Build history of the part. All positions in model axes, mm. A direction names the side the tool comes from. Round coordinates to 2 decimals unless told otherwise and drop trailing zeros. Write each loop counter-clockwise with the first axis right and the second up, starting at its lowest first coordinate (ties: lowest second). Pieces come first, ordered by that corner, then holes. Notation, with made-up numbers: (-4.5, 66) - (27.5, 66) arc R22 cw to (27.5, 95) - close; hole circle Ø8 at (12, 31.5). An arc over 180 degrees is marked (long way). Answer as a JSON object with one key per item and string values. Group by question number.
Item 1: Which spindle directions (+Z, -Z, +X, -X, +Y, -Y) get a long thin tool onto all of the face, cutting with end or side? Do faces 5 (the flat face through (-20, 2.686, 8)), 6 (the flat face through (20, 2.686, 8)), 7 (the cylindrical face through (23.959, -43.667, 7.395)). Say none if no direction does.
Item 2: Flat gauge pins, fed straight in: pin 1 (6.5 mm diameter, centred on x = -19.73, y = -42.81, fed in from -Z); pin 2 (1.2 mm diameter, centred on x = -19.5, z = 6, fed in from +Y); pin 3 (4 mm diameter, centred on x = 14, z = 11.5, fed in from -Y); pin 4 (4.5 mm diameter, centred on y = 19, z = 9, fed in from -X). Where does each tip first touch, or does it go through?
Item 3: Two-plate mould, pull along Y, no slides. Class faces 1 (the cylindrical face through (-1.96, 26.876, 10.563)), 2 (the cylindrical face through (-18.9, -38.9, 7.4)), 3 (the flat face through (-23.7, 1.21, 7.4)), 4 (the flat face through (-25.226, -22, 7)): +Y half, -Y half, draft (parallel to the pull), parting line (faces both ways), or undercut.
Item 4: Slice it at C-C, the plane x = 0. List the corners of the cut face in (y, z).
Item 5: Slice it at D-D, the plane y = -40.5. List the corners of the cut face in (x, z).
Item 6: Slice it at A-A, the plane y = 37. List the corners of the cut face in (x, z), then the cut area to 3 significant figures.
Item 7: Slice it at B-B, the plane z = 11.5. List the corners of the cut face in (x, y), then the cut area to 3 significant figures.
Item 8: Probe line 1 (Y direction, x = -17, z = 6.5); line 2 (Y direction, x = -2.5, z = 9); line 3 (X direction, y = 27.5, z = 3.25). List the from-to ranges inside material, lowest first. Write a range as from..to.
from build123d import *

# Parameters (mm, degrees)
SKETCH1_W           = 50
SKETCH1_H           = 97
BOSS_EXTRUDE1_DEPTH = 15
SKETCH6_R           = 8
CUT_EXTRUDE3_DEPTH  = 9
SKETCH7_R           = 4.5
CUT_EXTRUDE4_DEPTH  = 57.444472183
SKETCH8_R           = 20
SKETCH8_R_2         = 4
CUT_EXTRUDE5_DEPTH  = 58.705965376
SKETCH9_W           = 32.009633737
SKETCH9_H           = 62.03619176
SKETCH9_W_2         = 30.458131691
SKETCH9_H_2         = 52.571237354
CUT_EXTRUDE6_DEPTH  = 58.705965376
CHAMFER1_SIZE       = 3
SKETCH14_R          = 119.720313389
SKETCH14_R_2        = 82
CUT_EXTRUDE10_DEPTH = 58.705965376


with BuildPart() as part:
    # Sketch1 → Boss-Extrude1 (new body)
    with BuildSketch(Plane.XY):
        with Locations((-0.2255048, 1.185534591)):
            Rectangle(SKETCH1_W, SKETCH1_H)
    extrude(amount=BOSS_EXTRUDE1_DEPTH)

    # Sketch6 → Cut-Extrude3 (cut)
    with BuildSketch(Plane.XY.offset(15)):
        with Locations((-0.2255048, 34.685534591)):
            Circle(SKETCH6_R)
    extrude(amount=-CUT_EXTRUDE3_DEPTH, mode=Mode.SUBTRACT)

    # Sketch7 → Cut-Extrude4 (cut, through all)
    with BuildSketch(Plane.XY.offset(6)):
        with Locations((-0.2255048, 34.685534591)):
            Circle(SKETCH7_R)
    extrude(amount=-CUT_EXTRUDE4_DEPTH, mode=Mode.SUBTRACT)

    # Sketch8 → Cut-Extrude5 (cut, through all)
    with BuildSketch(Plane(origin=(0, 0, 0), x_dir=(-1, 0, 0), z_dir=(0, 0, -1))):
        with Locations((0.2255048, -23.314465409)):
            Circle(SKETCH8_R)
        with Locations((-19.2744952, -42.814465409)):
            Circle(SKETCH8_R_2)
        with Locations((-19.2744952, -3.814465409)):
            Circle(SKETCH8_R_2)
        with Locations((19.7255048, -3.814465409)):
            Circle(SKETCH8_R_2)
        with Locations((19.7255048, -42.814465409)):
            Circle(SKETCH8_R_2)
    extrude(amount=-CUT_EXTRUDE5_DEPTH, mode=Mode.SUBTRACT)

    # Sketch9 → Cut-Extrude6 (cut, through all)
    with BuildSketch(Plane.XY.offset(15)):
        with Locations((30.779312069, 33.703630471)):
            Rectangle(SKETCH9_W, SKETCH9_H)
        with Locations((-30.454570646, 28.971153268)):
            Rectangle(SKETCH9_W_2, SKETCH9_H_2)
    extrude(amount=-CUT_EXTRUDE6_DEPTH, mode=Mode.SUBTRACT)

    # Chamfer1
    chamfer1_edges = [part.edges().sort_by_distance(p)[0] for p in [
        (14.7744952, 49.685534591, 7.5),
        (14.7744952, 2.685534591, 7.5),
        (24.7744952, 2.685534591, 7.5),
        (-15.2255048, 49.685534591, 7.5),
        (-25.2255048, 2.685534591, 7.5),
        (-15.2255048, 2.685534591, 7.5),
    ]]
    chamfer(chamfer1_edges, length=CHAMFER1_SIZE)

    # Sketch14 → Cut-Extrude10 (cut, through all)
    with BuildSketch(Plane(origin=(0, 0, 0), x_dir=(-1, 0, 0), z_dir=(0, 0, -1))):
        with Locations((0.2255048, 34.685534591)):
            Circle(SKETCH14_R)
        with Locations((0.2255048, 34.685534591)):
            Circle(SKETCH14_R_2, mode=Mode.SUBTRACT)
    extrude(amount=-CUT_EXTRUDE10_DEPTH, mode=Mode.SUBTRACT)


solid = part.part
Geometry says:
{
 "1": {"face 5": "+Z, -Z, -X, +Y", "face 6": "+Z, -Z, +X, +Y", "face 7": "+Z, -Z, +X, -Y"},
 "2": {"pin 1": "passes through", "pin 2": "stops at y = 2.69", "pin 3": "stops at y = -46.4", "pin 4": "stops at x = -15.23"},
 "3": {"face 1": "undercut", "face 2": "undercut", "face 3": "+Y half", "face 4": "draft"},
 "4": {"outline": "(-47.31, 0) - (-43.31, 0) - (-43.31, 15) - (-47.31, 15) - close; (-3.32, 0) - (30.19, 0) - (30.19, 6) - (26.69, 6) - (26.69, 15) - (-3.32, 15) - close; (39.18, 0) - (49.69, 0) - (49.69, 15) - (42.68, 15) - (42.68, 6) - (39.18, 6) - close"},
 "5": {"outline": "(-25.23, 0) - (-22.99, 0) - (-22.99, 15) - (-25.23, 15) - close; (-16.46, 0) - (-10.46, 0) - (-10.46, 15) - (-16.46, 15) - close; (10, 0) - (16.01, 0) - (16.01, 15) - (10, 15) - close; (22.54, 0) - (24.77, 0) - (24.77, 15) - (22.54, 15) - close"},
 "6": {"outline": "(-15.23, 0) - (-4.08, 0) - (-4.08, 6) - (-7.88, 6) - (-7.88, 15) - (-15.23, 15) - close; (3.63, 0) - (14.77, 0) - (14.77, 15) - (7.43, 15) - (7.43, 6) - (3.63, 6) - close", "area": "266 mm^2"},
 "7": {"outline": "(-25.23, -43.41) arc R82 ccw to (-23.57, -43.92) arc R4 cw (long way) to (-16.86, -45.61) arc R82 ccw to (16.41, -45.61) arc R4 cw (long way) to (23.12, -43.92) arc R82 ccw to (24.77, -43.41) - (24.77, -0.31) - (21.77, 2.69) - (17.77, 2.69) - (14.77, 5.69) - (14.77, 46.69) - (11.77, 49.69) - (-12.23, 49.69) - (-15.23, 46.69) - (-15.23, 5.69) - (-18.23, 2.69) - (-22.23, 2.69) - (-25.23, -0.31) - close; hole circle Ø8 at (-19.73, -3.81); hole circle Ø40 at (-0.23, -23.31); hole circle Ø16 at (-0.23, 34.69); hole circle Ø8 at (19.27, -3.81)", "area": "2,200 mm^2"},
 "8": {"line 1": "y = -39.89..-34.21, -12.42..-6.74, -0.89..3.91", "line 2": "y = -47.28..-43.18, -3.44..27.02, 42.36..49.69", "line 3": "x = -15.23..14.77"}
}
